Check sheet for the modelled part. Datum: model origin and axes. Units: mm. A direction names the side the tool comes from. Coordinates: 2 decimals unless noted, no trailing zeros. Loops run counter-clockwise (first coordinate to the right, second up) from the corner with the lowest first, then second, coordinate; pieces in that order, holes last.
```python
from build123d import *

# Parameters (mm, degrees)
SKETCH1_W             = 35
SKETCH1_H             = 40
BOSS_EXTRUDE1_DEPTH   = 29
CHAMFER1_SIZE         = 20
M5_TAPPED_HOLE1_D     = 4.2
M5_TAPPED_HOLE1_DEPTH = 12.4
M5_TAPPED_HOLE1_TIP   = 1.2618073
M5_TAPPED_HOLE2_D     = 4.2
CHAMFER2_SIZE         = 2


with BuildPart() as part:
    # Sketch1 → Boss-Extrude1 (new body)
    with BuildSketch(Plane(origin=(0, 0, 0), x_dir=(1, 0, 0), z_dir=(0, 1, 0))):
        Rectangle(SKETCH1_W, SKETCH1_H)
    extrude(amount=BOSS_EXTRUDE1_DEPTH)

    # Chamfer1
    chamfer1_edges = [part.edges().sort_by_distance(p)[0] for p in [
        (0, 0, -20),
    ]]
    chamfer(chamfer1_edges, length=CHAMFER1_SIZE)

    # M5 Tapped Hole1
    with Locations(Plane(origin=(-10, 5.5, 20), x_dir=(1, 0, 0), z_dir=(0, 0, 1))):
        with Locations((0, 0), (20, 0)):
            Hole(M5_TAPPED_HOLE1_D / 2, depth=M5_TAPPED_HOLE1_DEPTH)
            with Locations((0, 0, -(M5_TAPPED_HOLE1_DEPTH + M5_TAPPED_HOLE1_TIP / 2))):  # 118° drill point
                Cone(0, M5_TAPPED_HOLE1_D / 2, M5_TAPPED_HOLE1_TIP, mode=Mode.SUBTRACT)

    # M5 Tapped Hole2 (through all)
    with Locations(Plane(origin=(-10, 29, -14), x_dir=(0, 0, 1), z_dir=(0, 1, 0))):
        with Locations((0, 0), (0, 20)):
            Hole(M5_TAPPED_HOLE2_D / 2)

    # Chamfer2
    chamfer2_edges = [part.edges().sort_by_distance(p)[0] for p in [
        (-17.5, 0, 10),
        (17.5, 0, 10),
    ]]
    chamfer(chamfer2_edges, length=CHAMFER2_SIZE)


solid = part.part
```
1) Section check B-B on z = 16. Enter the section's corners in (x, y), plus the area to 3 significant figures.
Answer sheet:
outline: (-17.5, 2) - (-15.5, 0) - (15.5, 0) - (17.5, 2) - (17.5, 29) - (-17.5, 29) - close; hole circle Ø4.2 at (-10, 5.5); hole circle Ø4.2 at (10, 5.5)
area: 983 mm2
2) Section check A-A on z = -14. Enter the section's corners in (x, y).
Answer sheet:
outline: (-17.5, 14) - (-12.1, 14) - (-12.1, 29) - (-17.5, 29) - close; (-7.9, 14) - (7.9, 14) - (7.9, 29) - (-7.9, 29) - close; (12.1, 14) - (17.5, 14) - (17.5, 29) - (12.1, 29) - close
3) Section check D-D on x = 4.5. Enter the section's corners in (y, z).
Answer sheet:
outline: (0, 0) - (20, -20) - (29, -20) - (29, 20) - (0, 20) - close
4) Section check C-C on y = 25. Enter the section's corners in (x, z).
Answer sheet:
outline: (-17.5, -20) - (17.5, -20) - (17.5, 20) - (-17.5, 20) - close; hole circle Ø4.2 at (-10, -14); hole circle Ø4.2 at (10, -14)
5) Scan lines: line 1 (X direction, y = 5.5, z = 10.5); line 2 (Z direction, x = 10, y = 25); line 3 (Y direction, x = 10, z = 15). Record each from-to range of solid material in increasing order.
Answer sheet:
line 1: x = -17.5 to -12.1, -7.9 to 7.9, 12.1 to 17.5
line 2: z = -20 to -16.1, -11.9 to 20
line 3: y = 0 to 3.4, 7.6 to 29
6) Depth check by flat-ended pin: pin 1 (2 mm diameter, centred on x = -10.5, y = 5.5, fed in from -Z); pin 2 (3.5 mm diameter, centred on x = -10, y = 5.5, fed in from +Z); pin 3 (1 mm diameter, centred on x = -8.5, y = 12, fed in from -Z). Enter the tip coordinate at first touch or a pass-through.
Answer sheet:
pin 1: stops at z = -6.5
pin 2: stops at z = 7.39
pin 3: stops at z = -12.5
7) Mould release check, pull along Z, two halves, no side actions. Record for faces 3 (the flat face through (16.5, 1, 9.2)), 4 (the conical face through (9.636, 5.516, 6.557)), 5 (the cylindrical face through (-9.91, 22.2, -11.9)): +Z half, -Z half, draft (parallel to the pull), parting line (faces both ways), or undercut.
Answer sheet:
face 3: draft
face 4: +Z half
face 5: undercut
8) Set-up check for faces 1 (the cylindrical face through (11.548, 6.919, 13.713)), 2 (the flat face through (0, 10, -10)): record each of +Z, -Z, +X, -X, +Y, -Y from which the full face is reachable in a straight line by a thin tool's end or side.
Answer sheet:
face 1: +Z
face 2: -Z, +X, -X, -Y
